Source: CAD feature listing. Evaluate the final solid. Frame: model axes, mm. A direction names the side the tool comes from. Give positions to 0.01 mm unless a question says otherwise; leave off trailing zeros. Order: outer loops, then holes, each group sorted by start corner. A loop starts at its lowest first (then second) coordinate and runs counter-clockwise, first axis right, second up. Notation, with made-up numbers: (-32.75, -29.75) - (20.25, -29.75) arc R20 ccw to (20.25, -0.75) - close; hole circle Ø10 at (81.25, 86.5). An arc over 180 degrees is marked (long way). Write each question's results on one line, items separated by ' | '. Start each with the question number.
Item 1: Section B-B on y = -27. Output: boundary loops of the cut face in (x, z), and give its area (3 significant figures).
Item 2: Section D-D on y = 11. Output: boundary loops of the cut face in (x, z), and give its area (3 significant figures).
Item 3: Mould query, pull axis Y, two halves, no side actions, for faces 1 (the cylindrical face through (-7.75, 28.19, -0.05)), 2 (the flat face through (0, -32.5, 0)), 3 (the cylindrical face through (20.412, 20.243, -2.739)). Classes: released by +Y, released by -Y, zero draft, split by the parting line, or undercut.
Item 4: Section A-A on x = 0. Output: boundary loops of the cut face in (y, z), and give its area (3 significant figures).
Item 5: Set-up query: faces 4 (the cylindrical face through (-27.57, 22.52, -0.33)), 5 (the flat face through (-3, -15, -2.4)), 6 (the cylindrical face through (27.57, 2.44, -0.54)). Return all of +Z, -Z, +X, -X, +Y, -Y with unobstructed straight access to the full face (end or side cutting, diameter ignored); none if empty.
Item 6: Line query: line 1 along Y through (x, z) = (-18, 0.25); line 2 along Y through (x, z) = (-28, 0); line 3 along X through (y, z) = (30, -1). Output: solid intervals per line, ascending.
Item 7: Section C-C on x = 28. Output: boundary loops of the cut face in (y, z).
Item 8: Contact query for flat-ended pins moving along their axis: pin 1 Ø1 at (y, z) = (0.5, -0.5) entering from -X; pin 2 Ø0.6 at (x, z) = (32, 1.5) entering from -Y; pin 3 Ø4.5 at (y, z) = (0, 0) entering from -X; pin 4 Ø5 at (x, y) = (-18.38, -18.38) entering from -Z. Output: stop coordinate, or through.
```python
from build123d import *

# Parameters (mm, degrees)
SKETCH_1_W                   = 65
SKETCH_1_H                   = 65
EXTRUDE_1_DEPTH              = 5.5
SKETCH_3_R                   = 20.05
CUT_EXTRUDE_1_DEPTH          = 3.1
SKETCH_4_R                   = 15
CUT_EXTRUDE_2_DEPTH          = 47.635930354
HOLE_WIZARD_M5_1_D           = 5.5
HOLE_WIZARD_M5_1_CBORE_D     = 10
HOLE_WIZARD_M5_1_CBORE_DEPTH = 5.4
HOLE_WIZARD_M6_1_AT_2_COUNT  = 2
HOLE_WIZARD_M6_1_AT_2_PITCH  = 25
SKETCH_12_W                  = 11
SKETCH_12_H                  = 10
SKETCH_12_H_2                = 25
CUT_EXTRUDE_3_DEPTH          = 0.5
CHAMFER_1_SIZE               = 2
HOLE_WIZARD_M3_2_D           = 2.5
HOLE_WIZARD_M3_2_DEPTH       = 8.5
HOLE_WIZARD_M3_2_TIP         = 0.751075774
HOLE_WIZARD_M3_3_D           = 2.5
HOLE_WIZARD_M3_3_DEPTH       = 8.5
HOLE_WIZARD_M3_3_TIP         = 0.751075774


with BuildPart() as part:
    # 草图1 → 凸台-拉伸1 (new, symmetric)
    with BuildSketch(Plane.XY):
        Rectangle(SKETCH_1_W, SKETCH_1_H)
    extrude(amount=EXTRUDE_1_DEPTH, both=True)

    # 草图3 → 切除-拉伸1 (cut)
    with BuildSketch(Plane(origin=(0, 0, -5.5), x_dir=(-1, 0, 0), z_dir=(0, 0, -1))):
        Circle(SKETCH_3_R)
    extrude(amount=-CUT_EXTRUDE_1_DEPTH, mode=Mode.SUBTRACT)

    # 草图4 → 切除-拉伸2 (cut, through all)
    with BuildSketch(Plane(origin=(0, 0, -2.4), x_dir=(-1, 0, 0), z_dir=(0, 0, -1))):
        Circle(SKETCH_4_R)
    extrude(amount=-CUT_EXTRUDE_2_DEPTH, mode=Mode.SUBTRACT)

    # M5 六角凹头螺钉的柱形沉头孔1 (through all)
    with Locations(Plane.XY.offset(5.5)):
        with Locations((-18.384776311, 18.384776311), (18.384776311, 18.384776311), (18.384776311, -18.384776311), (-18.384776311, -18.384776311)):
            CounterBoreHole(HOLE_WIZARD_M5_1_D / 2, HOLE_WIZARD_M5_1_CBORE_D / 2, HOLE_WIZARD_M5_1_CBORE_DEPTH)

    # 草图8 → M6 螺纹孔1 (revolve, cut)
    with BuildSketch(Plane(origin=(-32.5, 0, 0), x_dir=(0, 0, 1), z_dir=(0, 1, 0))):
        Polygon((0, 0), (0, 11.502151548), (2.5, 10), (2.5, 0), align=None)
    hole_wizard_m6_1 = revolve(axis=Axis((-38.85, 0, 0), (1, 0, 0)), mode=Mode.SUBTRACT)

    # M6 螺纹孔1 at 2: M6 螺纹孔1 ×2
    with Locations(*[(0, i * HOLE_WIZARD_M6_1_AT_2_PITCH, 0) for i in range(1, HOLE_WIZARD_M6_1_AT_2_COUNT)]):
        add(hole_wizard_m6_1, mode=Mode.SUBTRACT)

    # 草图12 → 切除-拉伸3 (cut)
    with BuildSketch(Plane.ZY.offset(32.5)):
        with Locations((0, 12.5)):
            Rectangle(SKETCH_12_W, SKETCH_12_H)
        with Locations((0, -20)):
            Rectangle(SKETCH_12_W, SKETCH_12_H_2)
    cut_extrude_3 = extrude(amount=-CUT_EXTRUDE_3_DEPTH, mode=Mode.SUBTRACT)

    # 镜向1: M6 螺纹孔1, 切除-拉伸3 across plane
    add(hole_wizard_m6_1.mirror(Plane(origin=(0, 0, 0), x_dir=(0, 0, 1), z_dir=(1, 0, 0))), mode=Mode.SUBTRACT)
    add(cut_extrude_3.mirror(Plane(origin=(0, 0, 0), x_dir=(0, 0, 1), z_dir=(1, 0, 0))), mode=Mode.SUBTRACT)

    # 镜向1 copy 1 sketch → 镜向1 copy 1 (revolve, cut)
    with BuildSketch(Plane(origin=(32.5, 25, 0), x_dir=(0, 0, 1), z_dir=(0, 1, 0))):
        Polygon((0, 0), (0, -11.502151548), (2.5, -10), (2.5, 0), align=None)
    revolve(axis=Axis((38.85, 25, 0), (1, 0, 0)), mode=Mode.SUBTRACT)

    # 倒角1
    chamfer_1_edges = [part.edges().sort_by_distance(p)[0] for p in [
        (32, -32.5, 0),
        (-32.5, 32.5, 0),
        (32.5, 32.5, 0),
        (-32, -32.5, 0),
    ]]
    chamfer(chamfer_1_edges, length=CHAMFER_1_SIZE)

    # M3 螺纹孔2
    with Locations(Plane(origin=(0, 32.5, 0), x_dir=(1, 0, 0), z_dir=(0, 1, 0))):
        with Locations((-9, 0), (9, 0)):
            Hole(HOLE_WIZARD_M3_2_D / 2, depth=HOLE_WIZARD_M3_2_DEPTH)
            with Locations((0, 0, -(HOLE_WIZARD_M3_2_DEPTH + HOLE_WIZARD_M3_2_TIP / 2))):  # 118° drill point
                Cone(0, HOLE_WIZARD_M3_2_D / 2, HOLE_WIZARD_M3_2_TIP, mode=Mode.SUBTRACT)

    # M3 螺纹孔3
    with Locations(Plane(origin=(0, -32.5, 0), x_dir=(-1, 0, 0), z_dir=(0, -1, 0))):
        with Locations((-9, 1.25), (9, 1.25)):
            Hole(HOLE_WIZARD_M3_3_D / 2, depth=HOLE_WIZARD_M3_3_DEPTH)
            with Locations((0, 0, -(HOLE_WIZARD_M3_3_DEPTH + HOLE_WIZARD_M3_3_TIP / 2))):  # 118° drill point
                Cone(0, HOLE_WIZARD_M3_3_D / 2, HOLE_WIZARD_M3_3_TIP, mode=Mode.SUBTRACT)


solid = part.part
```
Evaluation:
1) outline: (-32, -5.5) - (32, -5.5) - (32, 5.5) - (-32, 5.5) - close; hole circle Ø2.5 at (-9, -1.25); hole circle Ø2.5 at (9, -1.25) | area: 694 mm^2
2) outline: (-32, -5.5) - (-16.76, -5.5) - (-16.76, -2.4) - (-10.2, -2.4) - (-10.2, 5.5) - (-32, 5.5) - close; (10.2, -2.4) - (16.76, -2.4) - (16.76, -5.5) - (32, -5.5) - (32, 5.5) - (10.2, 5.5) - close | area: 439 mm^2
3) face 1: zero draft | face 2: released by -Y | face 3: undercut
4) outline: (-32.5, -5.5) - (-20.05, -5.5) - (-20.05, -2.4) - (-15, -2.4) - (-15, 5.5) - (-32.5, 5.5) - close; (15, -2.4) - (20.05, -2.4) - (20.05, -5.5) - (32.5, -5.5) - (32.5, 5.5) - (15, 5.5) - close | area: 354 mm^2
5) face 4: -X | face 5: -Z | face 6: +X
6) line 1: y = -32.5 to -23.37, -13.4 to 13.4, 23.37 to 32.5 | line 2: y = -32.5 to -2.5, 2.5 to 22.5, 27.5 to 32.5 | line 3: x = -32.5 to -9.75, -8.25 to 8.25, 9.75 to 32.5
7) outline: (-32.5, -5.5) - (32.5, -5.5) - (32.5, 5.5) - (-32.5, 5.5) - close; hole circle Ø5 at (0, 0); hole circle Ø5 at (25, 0)
8) pin 1: stops at x = -21.72 | pin 2: stops at y = -30.8 | pin 3: stops at x = -22.35 | pin 4: passes through
